from build123d import *

# Parameters (mm, degrees)
EXTRUDE_1_DEPTH     = 149
SKETCH_2_R          = 35
EXTRUDE_2_DEPTH     = 7
SKETCH_4_W          = 80
SKETCH_4_H          = 80
EXTRUDE_3_DEPTH     = 8
SKETCH_5_R          = 3
CUT_EXTRUDE_1_DEPTH = 8
FILLET_1_R          = 5
SKETCH_6_R          = 9.5
EXTRUDE_4_DEPTH     = 28
SKETCH_7_W          = 6
SKETCH_7_H          = 7.374792238
EXTRUDE_5_DEPTH     = 22
SKETCH_8_R          = 3
CUT_EXTRUDE_2_DEPTH = 34


with BuildPart() as part:
    # 草图1 → 凸台-拉伸1 (new body)
    with BuildSketch(Plane.XY):
        Polygon((25, 80), (0, 55), (0, 25), (25, 0), (55, 0), (80, 25), (80, 55), (55, 80), align=None)
    extrude(amount=EXTRUDE_1_DEPTH)

    # 草图2 → 凸台-拉伸2 (add)
    with BuildSketch(Plane.XY.offset(149)):
        with Locations((40, 40)):
            Circle(SKETCH_2_R)
    extrude(amount=EXTRUDE_2_DEPTH)

    # 草图4 → 凸台-拉伸3 (add)
    with BuildSketch(Plane.XY.offset(149)):
        with Locations((40, 40)):
            Rectangle(SKETCH_4_W, SKETCH_4_H)
    extrude(amount=-EXTRUDE_3_DEPTH)

    # 草图5 → 切除-拉伸1 (cut)
    with BuildSketch(Plane.XY.offset(149)):
        with Locations((8.180194847, 71.819805153)):
            Circle(SKETCH_5_R)
        with Locations((71.819805153, 71.819805153)):
            Circle(SKETCH_5_R)
        with Locations((71.819805153, 8.180194847)):
            Circle(SKETCH_5_R)
        with Locations((8.180194847, 8.180194847)):
            Circle(SKETCH_5_R)
    extrude(amount=-CUT_EXTRUDE_1_DEPTH, mode=Mode.SUBTRACT)

    # 圆角1
    fillet_1_edges = [part.edges().sort_by_distance(p)[0] for p in [
        (0, 0, 145),
        (80, 0, 145),
        (0, 80, 145),
        (80, 80, 145),
    ]]
    fillet(fillet_1_edges, radius=FILLET_1_R)

    # 草图6 → 凸台-拉伸4 (add)
    with BuildSketch(Plane.XY.offset(156)):
        with Locations((40, 40)):
            Circle(SKETCH_6_R)
    extrude(amount=EXTRUDE_4_DEPTH)


with BuildPart() as body_2:
    # 草图7 → 凸台-拉伸5 (new body)
    with BuildSketch(Plane.XY.offset(184)):
        with Locations((40, 49.687396119)):
            Rectangle(SKETCH_7_W, SKETCH_7_H)
    extrude(amount=-EXTRUDE_5_DEPTH)


with BuildPart() as part_1:
    add(part.part)

    # Combine 1: cut body 2
    add(body_2.part, mode=Mode.SUBTRACT)

    # 草图8 → 切除-拉伸2 (cut)
    with BuildSketch(Plane(origin=(0, 80, 0), x_dir=(1, 0, 0), z_dir=(0, 1, 0))):
        with Locations((40, -162)):
            Circle(SKETCH_8_R)
    extrude(amount=-CUT_EXTRUDE_2_DEPTH, mode=Mode.SUBTRACT)


solid = part_1.part
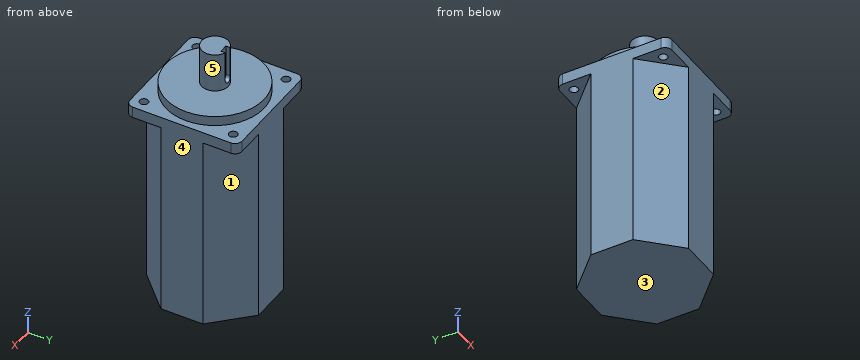
Input: part model. Units: mm. Frame: model coordinates. Face numbers are marked on the shaded views. A direction names the side the tool comes from. Give positions to 0.01 mm unless a question says otherwise; leave off trailing zeros. Loops run counter-clockwise (first coordinate to the right, second up) from the corner with the lowest first, then second, coordinate; pieces in that order, holes last. Notation, with made-up numbers: (63, 54.25) -> (103, 54.25) arc R25 ccw to (103, 72.25) -> close; hole circle Ø11 at (60.25, -12.75). An arc over 180 degrees is marked (long way). Answer as a JSON object with one key per item and string values. Group by question number.
Item 1: Cut plane A-A, the plane z = 138.5. Return the cut outline in (x, y), and give its area (3 significant figures).
Item 2: Line query: probe 1 along Z at (x, y) = (55, 64); probe 2 along X at (y, z) = (40, 164); probe 3 along Z at (x, y) = (5, 26.5). Output: solid intervals per line, ascending.
Item 3: Cut plane B-B, the plane x = 40. Return the cut outline in (y, z).
Item 4: Cut plane C-C, the plane y = 40. Return the cut outline in (x, z), and give its area (3 significant figures).
Item 5: Cut plane D-D, the plane y = 14. Return the cut outline in (x, z).
Item 6: Reachability of the marked faces 1, 2, 3, 4 and 5 from +Z, -Z, +X, -X, +Y, -Y: full face, straight path, thin tool, end or side. Return the list, or none.
Item 7: Pin query (flat end, axial travel): P1, Ø5, axis at x = 44.5, y = 56, coming from the +Z side; P2, Ø7, axis at x = 71.82, y = 8.18, coming from the +Z side; P3, Ø1.5, axis at y = 48, z = 167.5, coming from the -X side; P4, Ø5, axis at x = 46.5, y = 53, coming from the -Z side. Return the tip coordinate at first contact, or that it passes through.
Checks:
{
 "1": {"outline": "(0, 25) -> (25, 0) -> (55, 0) -> (80, 25) -> (80, 55) -> (55, 80) -> (25, 80) -> (0, 55) -> close", "area": "5,150 mm²"},
 "2": {"probe 1": "z = 0 to 156", "probe 2": "x = 30.5 to 49.5", "probe 3": "z = 0 to 149"},
 "3": {"outline": "(0, 0) -> (80, 0) -> (80, 149) -> (75, 149) -> (75, 156) -> (49.5, 156) -> (49.5, 159) -> (46, 159) -> (46, 184) -> (30.5, 184) -> (30.5, 156) -> (5, 156) -> (5, 149) -> (0, 149) -> close"},
 "4": {"outline": "(0, 0) -> (80, 0) -> (80, 149) -> (75, 149) -> (75, 156) -> (49.5, 156) -> (49.5, 184) -> (30.5, 184) -> (30.5, 156) -> (5, 156) -> (5, 149) -> (0, 149) -> close", "area": "12,900 mm²"},
 "5": {"outline": "(0, 141) -> (11, 141) -> (11, 0) -> (69, 0) -> (69, 141) -> (80, 141) -> (80, 149) -> (63.43, 149) -> (63.43, 156) -> (16.57, 156) -> (16.57, 149) -> (0, 149) -> close"},
 "6": {"face 1": "-Z, +X, +Y", "face 2": "-Z, -X, -Y", "face 3": "-Z, +X, -X, +Y, -Y", "face 4": "+Z, -Z, +X, +Y, -Y", "face 5": "+Z"},
 "7": {"P1": "stops at z = 156", "P2": "stops at z = 149", "P3": "stops at x = 33.86", "P4": "stops at z = 0"}
}
